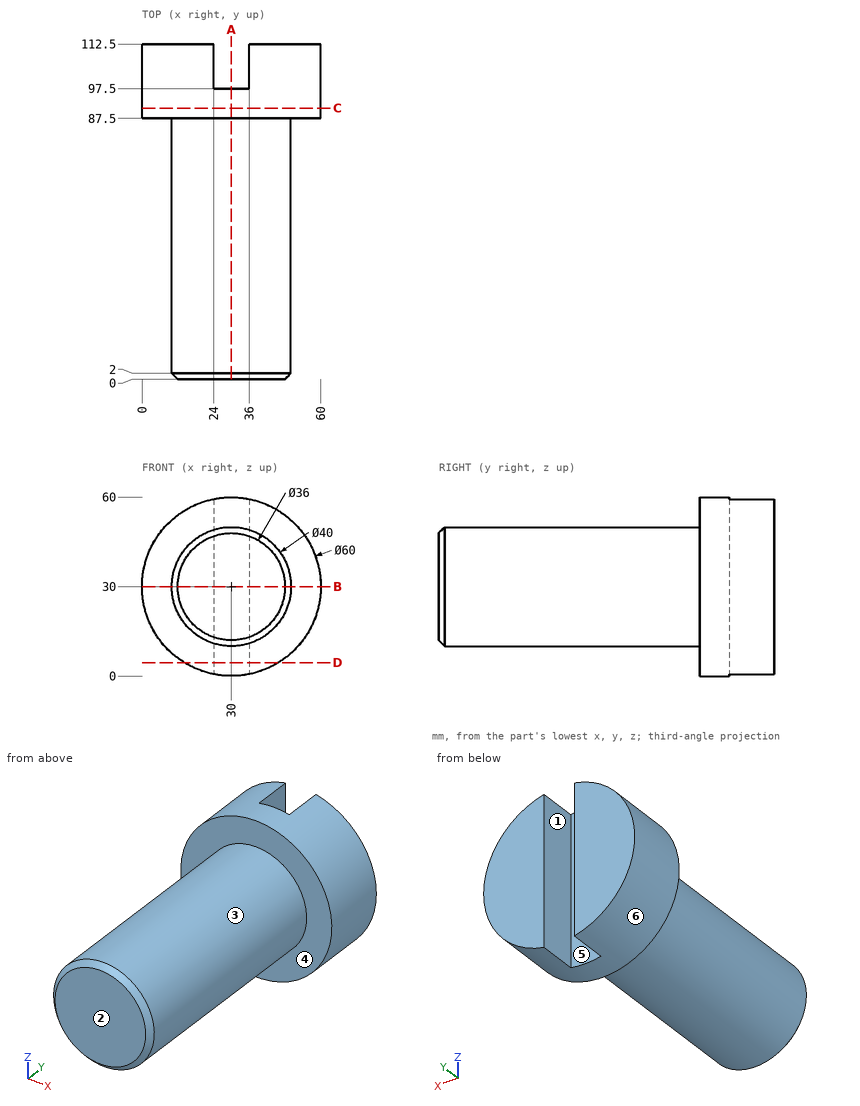
Can you work these out from the drawing? Everything is in mm from the part's minimum corner. A direction names the side the tool comes from. Round coordinates to 2 decimals unless told otherwise and drop trailing zeros. Order: outer loops, then holes, each group sorted by start corner. A loop starts at its lowest first (then second) coordinate and runs counter-clockwise, first axis right, second up. Notation, with made-up numbers: M 83,84 L 98,84 A10 cw 98,88 Z; hole C -31.5,-35.75 d10. An arc over 180 degrees is marked long. Answer as CSV lines item,"result".
Item 1: Imagine slicing it at B-B on z = 30. List the corners of the cut face in (x, y) for me, and give its area (3 significant figures).
From the geometry:
outline,"M 0,87.5 L 10,87.5 L 10,2 L 12,0 L 48,0 L 50,2 L 50,87.5 L 60,87.5 L 60,112.5 L 36,112.5 L 36,97.5 L 24,97.5 L 24,112.5 L 0,112.5 Z"
area,"4,820 mm2"
Item 2: Imagine slicing it at D-D on z = 4.5. List the corners of the cut face in (x, y) for me.
From the geometry:
outline,"M 14.2,87.5 L 45.8,87.5 L 45.8,112.5 L 36,112.5 L 36,97.5 L 24,97.5 L 24,112.5 L 14.2,112.5 Z"
Item 3: For pin 1 (6 mm diameter, centred on x = 30, z = 17, fed in from +Y); pin 2 (6 mm diameter, centred on x = 8, z = 13.5, fed in from -Y); pin 3 (12 mm diameter, centred on y = 102.5, z = 37.5, fed in from -X); pin 4 (5 mm diameter, centred on x = 7, y = 84.5, fed in from +Z), each with a flat end and sliding along its axis, tell me the tip position at first contact or that it passes through.
From the geometry:
pin 1,"y = 97.5"
pin 2,"y = 87.5"
pin 3,"x = 0.04"
pin 4,"through"
Item 4: Please list where these lines run through material, in increasing order: L1, parallel to X at y = 99.5, z = 31; L2, parallel to Y at x = 8, z = 48; L3, parallel to X at y = 101.5, z = 25. Write a range as [from, to].
From the geometry:
L1,"[0.02, 24], [36, 59.98]"
L2,"[87.5, 112.5]"
L3,"[0.42, 24], [36, 59.58]"
Item 5: We'd pull the mould along X, two halves only. Please class the marked faces 4, 5 and 6: +X half, -X half, draft (parallel to the pull), parting line (faces both ways), or undercut.
From the geometry:
face 4,"draft"
face 5,"undercut"
face 6,"parting line"
Item 6: Imagine slicing it at C-C on y = 91. List the corners of the cut face in (x, z) for me.
From the geometry:
outline,"C 30,30 d60"
Item 7: Imagine slicing it at A-A on x = 30. List the corners of the cut face in (y, z) for me, and give its area (3 significant figures).
From the geometry:
outline,"M 0,12 L 2,10 L 87.5,10 L 87.5,0 L 97.5,0 L 97.5,60 L 87.5,60 L 87.5,50 L 2,50 L 0,48 Z"
area,"4,100 mm2"
Item 8: Which directions (+Z, -Z, +X, -X, +Y, -Y) give clear straight access to the entire face, cutting with the end or side of a thin tool? Please do the marked faces 1, 2 and 3.
From the geometry:
face 1,"+Z, -Z, +Y"
face 2,"+Z, -Z, +X, -X, -Y"
face 3,"-Y"
